```python
from build123d import *

# Parameters (mm, degrees)
SKETCH_1_W                = 12
SKETCH_1_H                = 20
EXTRUDE_1_DEPTH           = 15
HOLE_WIZARD_1_D           = 4.5
HOLE_WIZARD_1_DEPTH       = 20
HOLE_WIZARD_1_CBORE_D     = 8
HOLE_WIZARD_1_CBORE_DEPTH = 4.6
HOLE_WIZARD_1_TIP         = 1.351936393
CHAMFER_1_SIZE            = 0.5


with BuildPart() as part:
    # 草图1 → 凸台-拉伸1 (new body)
    with BuildSketch(Plane(origin=(0, 0, 0), x_dir=(1, 0, 0), z_dir=(0, 1, 0))):
        Rectangle(SKETCH_1_W, SKETCH_1_H)
    extrude(amount=EXTRUDE_1_DEPTH)

    # 打孔尺寸(%根据)内六角圆柱头螺钉的类型1
    with Locations(Plane(origin=(0, 15, 0), x_dir=(1, 0, 0), z_dir=(0, 1, 0))):
        with Locations((0, 5), (0, -5)):
            CounterBoreHole(HOLE_WIZARD_1_D / 2, HOLE_WIZARD_1_CBORE_D / 2, HOLE_WIZARD_1_CBORE_DEPTH, depth=HOLE_WIZARD_1_DEPTH)
            with Locations((0, 0, -(HOLE_WIZARD_1_DEPTH + HOLE_WIZARD_1_TIP / 2))):  # 118° drill point
                Cone(0, HOLE_WIZARD_1_D / 2, HOLE_WIZARD_1_TIP, mode=Mode.SUBTRACT)

    # 倒角1
    chamfer_1_edges = [part.edges().sort_by_distance(p)[0] for p in [
        (6, 7.5, 10),
        (-6, 7.5, 10),
        (-6, 7.5, -10),
        (6, 7.5, -10),
    ]]
    chamfer(chamfer_1_edges, length=CHAMFER_1_SIZE)


solid = part.part
```
Geometry check sheet. Reference: the model listing, model coordinates, mm. A direction names the side the tool comes from. Give positions to 0.01 mm unless a question says otherwise; leave off trailing zeros. Order: outer loops, then holes, each group sorted by start corner. A loop starts at its lowest first (then second) coordinate and runs counter-clockwise, first axis right, second up. Notation, with made-up numbers: (16, -3.75) - (48, -3.75) arc R29 cw to (48, 35.25) - close; hole circle Ø9 at (-28, 22.25). An arc over 180 degrees is marked (long way). Answer in a Markdown table with one row per item. Add a question column.
Q1. Gauge pin test, flat ends, axial feed: pin 1 (4 mm diameter, centred on x = -1, z = 4.5, fed in from +Y); pin 2 (6.5 mm diameter, centred on x = 0, z = -5, fed in from -Y); pin 3 (3.5 mm diameter, centred on x = 0, z = -5, fed in from -Y). Record the tip position at first contact, or that the pin passes through.
Q2. Cross-section at C-C, the plane z = -4. Enter the section's corners in (x, y), then the cut area to 3 significant figures.
Q3. Cross-section at A-A, the plane x = 0. Enter the section's corners in (y, z).
Q4. Cross-section at D-D, the plane y = 9.25. Enter the section's corners in (x, z).
Q5. Material ranges on probe 1 along Z at (x, y) = (0, 3.75); probe 2 along Z at (x, y) = (0, 13); probe 3 along X at (y, z) = (2, -7), recorded low to high. Write a range as from..to.
Q6. Mould release check, pull along X, two halves, no side actions. Record for faces 3 (the flat face through (0, 15, 0)), 4 (the flat face through (6, 7, 0)), 5 (the cylindrical face through (0.488, 5.127, 7.196)), 6 (the flat face through (-6, 7, 0)): pulls with the +X half, pulls with the -X half, needs draft (parallel to the pull), parting line crosses it, or undercut.
Q7. Cross-section at B-B, the plane y = 14. Enter the section's corners in (x, z), then the cut area to 3 significant figures.
Q8. Tool access check on faces 1 (the cylindrical face through (0.29, 5.13, -7.23)), 2 (the flat face through (2, 10.4, 7)). Record the directions out of +Z, -Z, +X, -X, +Y, -Y that give a thin tool (end or side, any length) a straight path to the whole face; none if there is none.
Check values:
| question | item | result |
|---|---|---|
| 1 | pin 1 | stops at y = 10.4 |
| 1 | pin 2 | stops at y = 0 |
| 1 | pin 3 | passes through |
| 2 | outline | (-6, 0) - (-2.02, 0) - (-2.02, 10.4) - (-3.87, 10.4) - (-3.87, 15) - (-6, 15) - close; (2.02, 0) - (6, 0) - (6, 15) - (3.87, 15) - (3.87, 10.4) - (2.02, 10.4) - close |
| 2 | area | 102 mm^2 |
| 3 | outline | (0, -10) - (15, -10) - (15, -9) - (10.4, -9) - (10.4, -7.25) - (0, -7.25) - close; (0, -2.75) - (10.4, -2.75) - (10.4, -1) - (15, -1) - (15, 1) - (10.4, 1) - (10.4, 2.75) - (0, 2.75) - close; (0, 7.25) - (10.4, 7.25) - (10.4, 9) - (15, 9) - (15, 10) - (0, 10) - close |
| 4 | outline | (-6, -9.5) - (-5.5, -10) - (5.5, -10) - (6, -9.5) - (6, 9.5) - (5.5, 10) - (-5.5, 10) - (-6, 9.5) - close; hole circle Ø4.5 at (0, -5); hole circle Ø4.5 at (0, 5) |
| 5 | probe 1 | z = -10..-7.25, -2.75..2.75, 7.25..10 |
| 5 | probe 2 | z = -10..-9, -1..1, 9..10 |
| 5 | probe 3 | x = -6..-1.03, 1.03..6 |
| 6 | face 3 | needs draft |
| 6 | face 4 | pulls with the +X half |
| 6 | face 5 | undercut |
| 6 | face 6 | pulls with the -X half |
| 7 | outline | (-6, -9.5) - (-5.5, -10) - (5.5, -10) - (6, -9.5) - (6, 9.5) - (5.5, 10) - (-5.5, 10) - (-6, 9.5) - close; hole circle Ø8 at (0, -5); hole circle Ø8 at (0, 5) |
| 7 | area | 139 mm^2 |
| 8 | face 1 | +Y, -Y |
| 8 | face 2 | +Y |
